Can you work these out from the model? Positions are in its coordinate system, mm. Coordinates: 2 decimals unless noted, no trailing zeros. Loops run counter-clockwise (first coordinate to the right, second up) from the corner with the lowest first, then second, coordinate; pieces in that order, holes last. Notation, with made-up numbers: M 56.5,35 L 78.5,35 A22 ccw 78.5,61 Z; hole C 17,17 d3. An arc over 180 degrees is marked long. Answer as a JSON object with one key per item and string values. Group by question number.
Item 1: Suppose I cut it at B-B (y = 1.5). Write out the boundary of the cut face in (x, z), then the cut area to 4 significant figures.
Item 2: Suppose I cut it at A-A (x = 45). Write out the boundary of the cut face in (y, z), then the cut area to 3 significant figures.
Item 3: Suppose I cut it at C-C (z = -10.5). Write out the boundary of the cut face in (x, y).
Item 4: If I drill on line 1 (Y direction, x = 45, z = 9); line 2 (X direction, y = 1.5, z = -1); line 3 (X direction, y = 0.75, z = 0.5), over which ranges is the centre line in solid material (lowest first)?
```python
from build123d import *

# Parameters (mm, degrees)
PLATE_PROFILE_SKETCH_W          = 100
PLATE_PROFILE_SKETCH_H          = 12
BASE_PLATE_100X12X45_DEPTH      = 22.5
THROUGH_SLOT_AND_HOLE_CUT_REACH = 69.535
SLOT_AND_HOLE_SKETCH_R          = 2.5


with BuildPart() as part:
    # Plate Profile Sketch → Base Plate 100x12x45 (new, symmetric)
    with BuildSketch(Plane.XY):
        Rectangle(PLATE_PROFILE_SKETCH_W, PLATE_PROFILE_SKETCH_H)
    extrude(amount=BASE_PLATE_100X12X45_DEPTH, both=True)

    # Slot and Hole Sketch → Through Slot and Hole Cut (cut, up to next)
    with BuildSketch(Plane.XY.offset(22.5), mode=Mode.PRIVATE) as through_slot_and_hole_cut_sk1:
        with Locations((45, 0)):
            Circle(SLOT_AND_HOLE_SKETCH_R)
    through_slot_and_hole_cut_tool1 = extrude(through_slot_and_hole_cut_sk1.sketch, amount=-THROUGH_SLOT_AND_HOLE_CUT_REACH, mode=Mode.PRIVATE) & part.part
    # Slot and Hole Sketch → Through Slot and Hole Cut (cut, up to next)
    with BuildSketch(Plane.XY.offset(22.5), mode=Mode.PRIVATE) as through_slot_and_hole_cut_sk2:
        with BuildLine():
            Line((-45, 2.5), (-20, 2.5))
            ThreePointArc((-20, 2.5), (-17.5, 0), (-20, -2.5))
            Line((-20, -2.5), (-45, -2.5))
            ThreePointArc((-45, -2.5), (-47.5, 0), (-45, 2.5))
        make_face()
    through_slot_and_hole_cut_tool2 = extrude(through_slot_and_hole_cut_sk2.sketch, amount=-THROUGH_SLOT_AND_HOLE_CUT_REACH, mode=Mode.PRIVATE) & part.part
    add(through_slot_and_hole_cut_tool1.solids().sort_by_distance((45, 0, 22.5))[0], mode=Mode.SUBTRACT)
    add(through_slot_and_hole_cut_tool2.solids().sort_by_distance((-32.5, 0, 22.5))[0], mode=Mode.SUBTRACT)


solid = part.part
```
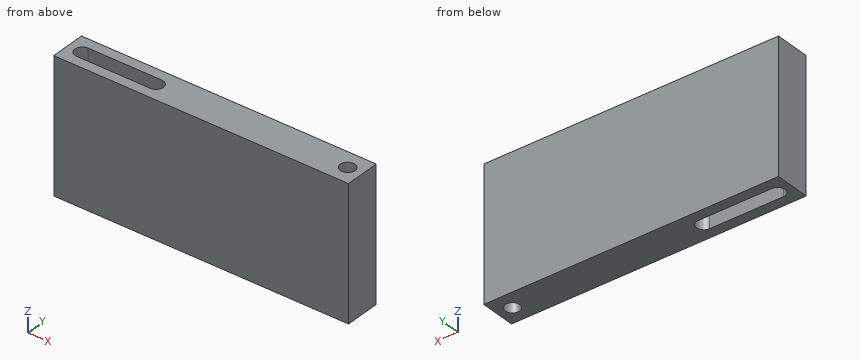
From the geometry:
{
 "1": {"outline": "M -50,-22.5 L -47,-22.5 L -47,22.5 L -50,22.5 Z; M -18,-22.5 L 43,-22.5 L 43,22.5 L -18,22.5 Z; M 47,-22.5 L 50,-22.5 L 50,22.5 L 47,22.5 Z", "area": "3,015 mm2"},
 "2": {"outline": "M -6,-22.5 L -2.5,-22.5 L -2.5,22.5 L -6,22.5 Z; M 2.5,-22.5 L 6,-22.5 L 6,22.5 L 2.5,22.5 Z", "area": "315 mm2"},
 "3": {"outline": "M -50,-6 L 50,-6 L 50,6 L -50,6 Z; hole M -45,-2.5 L -20,-2.5 A2.5 ccw -20,2.5 L -45,2.5 A2.5 ccw Z; hole C 45,0 d5"},
 "4": {"line 1": "-6 to -2.5, 2.5 to 6", "line 2": "-50 to -47, -18 to 43, 47 to 50", "line 3": "-50 to -47.38, -17.62 to 42.62, 47.38 to 50"}
}
